from build123d import *

# Parameters (mm, degrees)
SKETCH1_W             = 75
SKETCH1_H             = 7.5
CHAMFER3_SIZE         = 0.5
M6_TAPPED_HOLE1_D     = 5
M6_TAPPED_HOLE1_DEPTH = 15
M6_TAPPED_HOLE1_TIP   = 1.502151548
SKETCH7_R             = 10
BOSS_EXTRUDE2_DEPTH   = 15.5
CHAMFER4_SIZE         = 0.5
SKETCH8_OUTSIDE_W     = 38.032
SKETCH8_OUTSIDE_H     = 38.032
SKETCH8_OUTSIDE_W_2   = 25
SKETCH8_OUTSIDE_H_2   = 15
CUT_EXTRUDE1_DEPTH    = 62.15758334
SKETCH11_OUTSIDE_W    = 37.812
SKETCH11_OUTSIDE_H    = 32.812
SKETCH11_OUTSIDE_R    = 5.5
CUT_EXTRUDE2_DEPTH    = 5
CHAMFER5_SIZE         = 0.5


with BuildPart() as part:
    # Sketch1 → Revolve1 (revolve)
    with BuildSketch(Plane.XY, mode=Mode.PRIVATE) as revolve1_sk:
        with Locations((0, 3.75)):
            Rectangle(SKETCH1_W, SKETCH1_H)
    revolve(revolve1_sk.sketch.rotate(Axis((-37.5, 0, 0), (1, 0, 0)), 90), axis=Axis((-37.5, 0, 0), (1, 0, 0)))

    # Chamfer3
    chamfer3_edges = [part.edges().sort_by_distance(p)[0] for p in [
        (-37.5, 0, -7.5),
    ]]
    chamfer(chamfer3_edges, length=CHAMFER3_SIZE)

    # M6 Tapped Hole1
    with Locations(Plane.ZY.offset(37.5)):
        with Locations((0, 0)):
            Hole(M6_TAPPED_HOLE1_D / 2, depth=M6_TAPPED_HOLE1_DEPTH)
            with Locations((0, 0, -(M6_TAPPED_HOLE1_DEPTH + M6_TAPPED_HOLE1_TIP / 2))):  # 118° drill point
                Cone(0, M6_TAPPED_HOLE1_D / 2, M6_TAPPED_HOLE1_TIP, mode=Mode.SUBTRACT)

    # Sketch7 → Boss-Extrude2 (add)
    with BuildSketch(Plane(origin=(37.5, 0, 0), x_dir=(0, 0, -1), z_dir=(1, 0, 0))):
        Circle(SKETCH7_R)
    extrude(amount=-BOSS_EXTRUDE2_DEPTH)

    # Chamfer4
    chamfer4_edges = [part.edges().sort_by_distance(p)[0] for p in [
        (22, 0, 10),
        (37.5, 0, 10),
    ]]
    chamfer(chamfer4_edges, length=CHAMFER4_SIZE)

    # Sketch8 outside → Cut-Extrude1 (cut, through all)
    with BuildSketch(Plane.ZY.offset(-22)):
        Rectangle(SKETCH8_OUTSIDE_W, SKETCH8_OUTSIDE_H)
        Rectangle(SKETCH8_OUTSIDE_W_2, SKETCH8_OUTSIDE_H_2, mode=Mode.SUBTRACT)
    extrude(amount=-CUT_EXTRUDE1_DEPTH, mode=Mode.SUBTRACT)

    # Sketch11 outside → Cut-Extrude2 (cut)
    with BuildSketch(Plane.ZY.offset(37.5)):
        Rectangle(SKETCH11_OUTSIDE_W, SKETCH11_OUTSIDE_H)
        Circle(SKETCH11_OUTSIDE_R, mode=Mode.SUBTRACT)
    extrude(amount=-CUT_EXTRUDE2_DEPTH, mode=Mode.SUBTRACT)

    # Chamfer5
    chamfer5_edges = [part.edges().sort_by_distance(p)[0] for p in [
        (-37.5, 0, -5.5),
    ]]
    chamfer(chamfer5_edges, length=CHAMFER5_SIZE)


solid = part.part
Check sheet for the modelled part. Datum: model origin and axes. Units: mm. A direction names the side the tool comes from. Round coordinates to 2 decimals unless told otherwise and drop trailing zeros. Loops run counter-clockwise (first coordinate to the right, second up) from the corner with the lowest first, then second, coordinate; pieces in that order, holes last.
1. Sectioned sample at B-B on x = -26.5. Record the boundary of the cut face in (y, z), and give its area (3 significant figures).
2. Sectioned sample at A-A on x = 32. Record the boundary of the cut face in (y, z), and give its area (3 significant figures).
3. Scan lines: probe 1 along Y at (x, z) = (-33, 0); probe 2 along Y at (x, z) = (-28.5, 0); probe 3 along Z at (x, y) = (-24, 1.75). Record each from-to range of solid material in increasing order.
4. Set-up check for faces 5 (the cylindrical face through (-29.9, -2.44, 0.54)), 6 (the flat face through (37.5, 0, 0)), 7 (the flat face through (22, 0, -8)): record each of +Z, -Z, +X, -X, +Y, -Y from which the full face is reachable in a straight line by a thin tool's end or side.
5. Sectioned sample at C-C on x = 7. Record the boundary of the cut face in (y, z), and give its area (3 significant figures).
6. Gauge pin test, flat ends, axial feed: pin 1 Ø1.5 at (x, y) = (23, -2) entering from +Z; pin 2 Ø8 at (x, y) = (7.5, 4.5) entering from +Z; pin 3 Ø3 at (x, z) = (-19.5, -8) entering from +Y. Record the tip position at first contact, or that the pin passes through.
7. Mould release check, pull along Y, two halves, no side actions. Record for faces 1 (the flat face through (30, -7.5, 0)), 2 (the conical face through (-21, 0, 0)), 3 (the flat face through (22, -1, 8)), 4 (the cylindrical face through (-34.78, -5.37, -1.19)): released by +Y, released by -Y, zero draft, split by the parting line, or undercut.
Recorded:
1. outline: circle Ø15 at (0, 0); hole circle Ø5 at (0, 0)
1. area: 157 mm2
2. outline: (-7.5, -6.61) arc R10 ccw to (7.5, -6.61) - (7.5, 6.61) arc R10 ccw to (-7.5, 6.61) - close
2. area: 269 mm2
3. probe 1: y = -5.5 to -2.5, 2.5 to 5.5
3. probe 2: y = -7.5 to -2.5, 2.5 to 7.5
3. probe 3: z = -7.29 to -1.79, 1.79 to 7.29
4. face 5: -X
4. face 6: +Z, -Z, +X, +Y, -Y
4. face 7: -Z, -X
5. outline: circle Ø15 at (0, 0)
5. area: 177 mm2
6. pin 1: stops at z = 9.92
6. pin 2: stops at z = 7.48
6. pin 3: stops at y = 3.74
7. face 1: released by -Y
7. face 2: undercut
7. face 3: zero draft
7. face 4: split by the parting line
